Read the model definition and answer for the solid it produces. Units are mm, in the model's axes. Face numbers are marked on the shaded views. A direction names the side the tool comes from. Give positions to 0.01 mm unless a question says otherwise; leave off trailing zeros. Loops run counter-clockwise (first coordinate to the right, second up) from the corner with the lowest first, then second, coordinate; pieces in that order, holes last.
(1) Determine the mould class of the marked faces 3, 4, 5 and 6 for opening direction Z: pulls with the +Z half, pulls with the -Z half, needs draft (parallel to the pull), parting line crosses it, or undercut.
(2) Find section B-B, the plane x = -9.5. Write down the section's boundary in (y, z).
(3) Straight lines are drawn through the part: probe 1 along Y at (x, z) = (12, -54.5); probe 2 along Z at (x, y) = (3.5, 42.5); probe 3 along Y at (x, z) = (17, -33.5). For each, find the intervals that lie inside material, in ascending order.
(4) Each of these flat-tipped pins is pushed along its axis until it touches: P1, Ø5, axis at x = -2, z = -60.5, coming from the -Y side; P2, Ø6, axis at x = 15, y = 160, coming from the +Z side. Where does it stop, or does it pass through?
(5) Find section C-C, the plane y = 26. Write down the section's boundary in (x, z), then the cut area to 3 significant figures.
(6) Find section A-A, the plane z = -48. Write down the section's boundary in (x, y).
(7) Which of the six approach directions +Z, -Z, +X, -X, +Y, -Y give full straight-line access (tool end or side, diameter ignored) to the marked faces 1 and 2?
(8) Find section D-D, the plane z = -28. Write down the section's boundary in (x, y), then the cut area to 3 significant figures.
```python
from build123d import *

# Parameters (mm, degrees)
BOSS_EXTRUDE1_DEPTH = 20
CHAMFER1_SIZE       = 10


with BuildPart() as part:
    # Sketch1 → Boss-Extrude1 (new, symmetric)
    with BuildSketch(Plane(origin=(0, 0, 0), x_dir=(0, 0, -1), z_dir=(1, 0, 0))):
        Polygon((0, 0), (70, -35), (70, 194), (0, 194), align=None)
        with BuildLine():
            Line((32.5, 114), (32.5, 164))
            ThreePointArc((32.5, 164), (45, 176.5), (57.5, 164))
            Line((57.5, 164), (57.5, 114))
            ThreePointArc((57.5, 114), (45, 101.5), (32.5, 114))
        make_face(mode=Mode.SUBTRACT)
        with BuildLine():
            Line((32.5, 30.910324642), (32.5, 64))
            ThreePointArc((32.5, 64), (45, 76.5), (57.5, 64))
            Line((57.5, 64), (57.5, 30.910324642))
            ThreePointArc((57.5, 30.910324642), (45, 18.410324642), (32.5, 30.910324642))
        make_face(mode=Mode.SUBTRACT)
    extrude(amount=BOSS_EXTRUDE1_DEPTH, both=True)

    # Chamfer1
    chamfer1_edges = [part.edges().sort_by_distance(p)[0] for p in [
        (20, 79.5, -70),
        (20, 194, -35),
        (20, 97, 0),
        (20, -17.5, -35),
    ]]
    chamfer(chamfer1_edges, length=CHAMFER1_SIZE)


solid = part.part
```
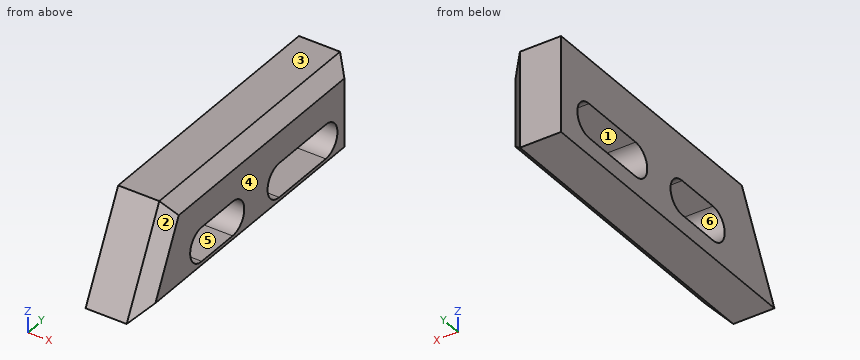
Entries:
1. face 3: pulls with the +Z half
1. face 4: needs draft
1. face 5: undercut
1. face 6: undercut
2. outline: (-35, -70) - (194, -70) - (194, 0) - (0, 0) - close; hole (30.91, -57.5) - (64, -57.5) arc R12.5 ccw to (64, -32.5) - (30.91, -32.5) arc R12.5 ccw to start; hole (114, -57.5) - (164, -57.5) arc R12.5 ccw to (164, -32.5) - (114, -32.5) arc R12.5 ccw to start
3. probe 1: y = -25.01 to 22.79, 72.12 to 105.88, 172.12 to 192
3. probe 2: z = -70 to -57.5, -32.5 to 0
3. probe 3: y = -8.92 to 26.01, 68.9 to 109.1, 168.9 to 187
4. P1: stops at y = -31.5
4. P2: stops at z = -2
5. outline: (-20, -70) - (10, -70) - (20, -60) - (20, -56.5) - (-20, -56.5) - close; (-20, -33.5) - (20, -33.5) - (20, -10) - (10, 0) - (-20, 0) - close
5. area: 1,780 mm2
6. outline: (-20, -24) - (10, -24) - (20, -12.82) - (20, 18.78) - (-20, 18.78) - close; (-20, 76.13) - (20, 76.13) - (20, 101.87) - (-20, 101.87) - close; (-20, 176.13) - (20, 176.13) - (20, 184) - (10, 194) - (-20, 194) - close
7. face 1: +X, -X
7. face 2: +Z, +X, -Y
8. outline: (-20, -14) - (10, -14) - (20, -2.82) - (20, 184) - (10, 194) - (-20, 194) - close
8. area: 8,210 mm2
